Read the model definition and answer for the solid it produces. Units are mm, in the model's axes. Coordinates: 2 decimals unless noted, no trailing zeros. Write each loop counter-clockwise with the first axis right and the second up, starting at its lowest first coordinate (ties: lowest second). Pieces come first, ordered by that corner, then holes.
1) The part is cut by section A-A (z = 0). Determine the outline of the cut face in (x, y).
2) The part is cut by section C-C (x = 6.25). Give the number of separate pieces and of enclosed holes in the cut face, then the cut area to 3 significant figures.
3) The part is cut by section B-B (y = -374). Determine the outline of the cut face in (x, z).
4) Each of these flat-tipped pins is pushed along its axis until it touches: pin 1 Ø2 at (x, y) = (2, -302.5) entering from +Z; pin 2 Ø1.5 at (x, z) = (2, 220.5) entering from -Y; pin 3 Ø8 at (x, y) = (8, -287.5) entering from -Z; pin 4 Ø21 at (y, z) = (0, -281) entering from -X. Where does it stop, or does it pass through?
5) Find the intervals of material crossed by line 1 (Y direction, x = 8.75, z = 0); line 2 (Y direction, x = 14, z = 253); line 3 (Z direction, x = 8.25, y = -375.5), in increasing order.
from build123d import *

# Parameters (mm, degrees)
SKETCH1_R           = 40.25
SKETCH1_R_2         = 45.25
SKETCH1_R_3         = 4.25
SKETCH1_R_4         = 3.5
SKETCH1_R_5         = 8
BOSS_EXTRUDE1_DEPTH = 16
FILLET1_R           = 20
SKETCH2_R           = 4.25
SKETCH2_R_2         = 3.5
BOSS_EXTRUDE2_DEPTH = 16


with BuildPart() as part:
    # Sketch1 → Boss-Extrude1 (new body)
    with BuildSketch(Plane(origin=(0, 0, 0), x_dir=(0, 0, -1), z_dir=(1, 0, 0))):
        with BuildLine():
            Line((-281, 20), (-221, 20))
            ThreePointArc((-221, 20), (-164.431457505, 43.431457505), (-141, 100))
            Line((-141, 100), (-141, 279))
            Line((-141, 279), (-100, 279))
            Line((-100, 279), (-100, 304))
            Line((-100, 304), (-68.44064835, 427.389656469))
            ThreePointArc((-68.44064835, 427.389656469), (-50.663636253, 454.493561649), (-20, 465))
            Line((-20, 465), (20, 465))
            ThreePointArc((20, 465), (50.663636253, 454.493561649), (68.44064835, 427.389656469))
            Line((68.44064835, 427.389656469), (100, 304))
            Line((100, 304), (100, 279))
            Line((100, 279), (141, 279))
            Line((141, 279), (141, 100))
            ThreePointArc((141, 100), (164.431457505, 43.431457505), (221, 20))
            Line((221, 20), (281, 20))
            ThreePointArc((281, 20), (301, 0), (281, -20))
            Line((281, -20), (221, -20))
            ThreePointArc((221, -20), (164.431457505, -43.431457505), (141, -100))
            Line((141, -100), (141, -279))
            Line((141, -279), (100, -279))
            Line((100, -279), (100, -304))
            Line((100, -304), (68.44064835, -427.389656469))
            ThreePointArc((68.44064835, -427.389656469), (50.663636253, -454.493561649), (20, -465))
            Line((20, -465), (-20, -465))
            ThreePointArc((-20, -465), (-50.663636253, -454.493561649), (-68.44064835, -427.389656469))
            Line((-68.44064835, -427.389656469), (-100, -304))
            Line((-100, -304), (-100, -279))
            Line((-100, -279), (-141, -279))
            Line((-141, -279), (-141, -100))
            ThreePointArc((-141, -100), (-164.431457505, -43.431457505), (-221, -20))
            Line((-221, -20), (-281, -20))
            ThreePointArc((-281, -20), (-301, 0), (-281, 20))
        make_face()
        with Locations((0, 374)):
            Circle(SKETCH1_R, mode=Mode.SUBTRACT)
        Circle(SKETCH1_R_2, mode=Mode.SUBTRACT)
        with Locations(Location((0, -374, 0), (0, 0, 180))):
            Circle(SKETCH1_R, mode=Mode.SUBTRACT)
        with Locations((20, -75)):
            Circle(SKETCH1_R_3, mode=Mode.SUBTRACT)
        with Locations((-20, -75)):
            Circle(SKETCH1_R_3, mode=Mode.SUBTRACT)
        with Locations((-20, 442)):
            Circle(SKETCH1_R_4, mode=Mode.SUBTRACT)
        with Locations((20, 442)):
            Circle(SKETCH1_R_4, mode=Mode.SUBTRACT)
        with Locations(Location((-20, -442, 0), (0, 0, 180))):
            Circle(SKETCH1_R_3, mode=Mode.SUBTRACT)
        with Locations(Location((20, -442, 0), (0, 0, 180))):
            Circle(SKETCH1_R_3, mode=Mode.SUBTRACT)
        with Locations((-281, 0)):
            Circle(SKETCH1_R_5, mode=Mode.SUBTRACT)
        with Locations((281, 0)):
            Circle(SKETCH1_R_5, mode=Mode.SUBTRACT)
    extrude(amount=BOSS_EXTRUDE1_DEPTH)

    # Fillet1
    fillet1_edges = [part.edges().sort_by_distance(p)[0] for p in [
        (8, 279, -141),
        (8, -279, -141),
        (8, -279, 141),
        (8, 279, 141),
    ]]
    fillet(fillet1_edges, radius=FILLET1_R)

    # Sketch2 → Boss-Extrude2 (add)
    with BuildSketch(Plane.ZY):
        with Locations((20, -442)):
            Circle(SKETCH2_R)
        with Locations((-20, -442)):
            Circle(SKETCH2_R)
        with Locations((20, -75)):
            Circle(SKETCH2_R)
        with Locations((-20, -75)):
            Circle(SKETCH2_R)
        with Locations((20, 442)):
            Circle(SKETCH2_R_2)
        with Locations((-20, 442)):
            Circle(SKETCH2_R_2)
    extrude(amount=-BOSS_EXTRUDE2_DEPTH)


solid = part.part
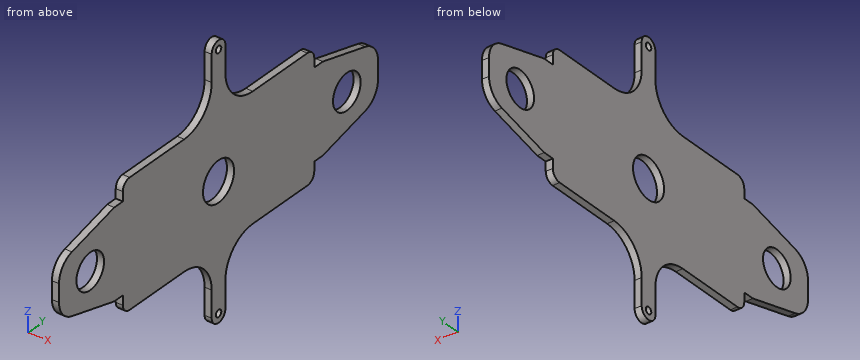
Reported:
1. outline: (0, -465) - (16, -465) - (16, -414.25) - (0, -414.25) - close; (0, -333.75) - (16, -333.75) - (16, -45.25) - (0, -45.25) - close; (0, 45.25) - (16, 45.25) - (16, 333.75) - (0, 333.75) - close; (0, 414.25) - (16, 414.25) - (16, 465) - (0, 465) - close
2. separate pieces: 1
2. enclosed holes: 5
2. area: 218,000 mm2
3. outline: (0, -82.1) - (16, -82.1) - (16, -40.25) - (0, -40.25) - close; (0, 40.25) - (16, 40.25) - (16, 82.1) - (0, 82.1) - close
4. pin 1: stops at z = 100
4. pin 2: stops at y = -20.01
4. pin 3: stops at z = -100
4. pin 4: stops at x = 0
5. line 1: y = -465 to -414.25, -333.75 to -45.25, 45.25 to 333.75, 414.25 to 465
5. line 2: y = -20 to 20
5. line 3: z = -81.71 to -40.22, 40.22 to 81.71
